Geometry check sheet. Reference: the model listing, model coordinates, mm. Face numbers are marked on the shaded views. A direction names the side the tool comes from. Round coordinates to 2 decimals unless told otherwise and drop trailing zeros. Loops run counter-clockwise (first coordinate to the right, second up) from the corner with the lowest first, then second, coordinate; pieces in that order, holes last. Notation, with made-up numbers: M -27,-34.75 L -12,-34.75 A28 cw -12,-7.75 Z; hole C 45,72.5 d3. An arc over 180 degrees is marked long. Write item = value, one per line.
from build123d import *

# Parameters (mm, degrees)
BOSS_EXTRUDE1_DEPTH                                  = 7.5
SKETCH2_W                                            = 168
SKETCH2_H                                            = 12
CUT_EXTRUDE1_DEPTH                                   = 12
CUT_EXTRUDE2_DEPTH                                   = 489.185415595
SKETCH4_W                                            = 22
SKETCH4_H                                            = 220
CUT_EXTRUDE3_DEPTH                                   = 1.5
F_11_0_11_DIAMETER_HOLE1_D                           = 11
F_11_0_11_DIAMETER_HOLE1_DEPTH                       = 30
SKETCH17_W                                           = 13.5
SKETCH17_H                                           = 16
CUT_EXTRUDE4_DEPTH                                   = 5
M6_TAPPED_HOLE2_D                                    = 5
M6_TAPPED_HOLE2_DEPTH                                = 15
M6_TAPPED_HOLE2_TIP                                  = 1.502151548
M4_TAPPED_HOLE1_D                                    = 3.3
M4_TAPPED_HOLE1_DEPTH                                = 10.1
M4_TAPPED_HOLE1_TIP                                  = 0.991420021
HOLE_SIZE_PER_SOCKET_HEAD_CAP_SCREW_TYPE_D           = 11
HOLE_SIZE_PER_SOCKET_HEAD_CAP_SCREW_TYPE_CBORE_D     = 18
HOLE_SIZE_PER_SOCKET_HEAD_CAP_SCREW_TYPE_CBORE_DEPTH = 11
F_10_0_10_DIAMETER_HOLE1_D                           = 10
F_10_0_10_DIAMETER_HOLE1_DEPTH                       = 30
F_10_0_10_DIAMETER_HOLE1_TIP                         = 3.004303095
M8_TAPPED_HOLE3_D                                    = 6.8
M8_TAPPED_HOLE3_DEPTH                                = 19.75
M8_TAPPED_HOLE3_TIP                                  = 2.042926105
M6_TAPPED_HOLE3_D                                    = 5
M6_TAPPED_HOLE3_DEPTH                                = 15
M6_TAPPED_HOLE3_TIP                                  = 1.502151548
FILLET1_R                                            = 5
M5_TAPPED_HOLE1_D                                    = 4.2
M5_TAPPED_HOLE1_DEPTH                                = 12.4
M5_TAPPED_HOLE1_TIP                                  = 1.2618073
CHAMFER1_SIZE                                        = 1
SKETCH36_OUTSIDE_W                                   = 449.638
SKETCH36_OUTSIDE_H                                   = 439.638
SKETCH36_OUTSIDE_W_2                                 = 200
SKETCH36_OUTSIDE_H_2                                 = 72
CUT_EXTRUDE6_DEPTH                                   = 489.185415598
M4_TAPPED_HOLE2_D                                    = 3.3
M4_TAPPED_HOLE2_DEPTH                                = 10.1
M4_TAPPED_HOLE2_TIP                                  = 0.991420021
HOLE_SIZE_PER_SOCKET_HEAD_CAP_SCREW_2_D              = 5.5
HOLE_SIZE_PER_SOCKET_HEAD_CAP_SCREW_2_CBORE_D        = 9.5
HOLE_SIZE_PER_SOCKET_HEAD_CAP_SCREW_2_CBORE_DEPTH    = 5.7
CHAMFER2_SIZE                                        = 2


with BuildPart() as part:
    # Sketch1 → Boss-Extrude1 (new, symmetric)
    with BuildSketch(Plane.XY):
        Polygon((0, 0), (0, 340), (168, 340), (168, 220), (350, 220), (350, 0), align=None)
    extrude(amount=BOSS_EXTRUDE1_DEPTH, both=True)

    # Sketch2 → Cut-Extrude1 (cut)
    with BuildSketch(Plane(origin=(0, 340, 0), x_dir=(1, 0, 0), z_dir=(0, 1, 0))):
        with Locations((84, 1.5)):
            Rectangle(SKETCH2_W, SKETCH2_H)
    extrude(amount=-CUT_EXTRUDE1_DEPTH, mode=Mode.SUBTRACT)

    # Sketch3 → Cut-Extrude2 (cut, through all)
    with BuildSketch(Plane.XY.offset(7.5)):
        with BuildLine():
            Line((45, 110), (135, 110))
            ThreePointArc((135, 110), (138.535533906, 108.535533906), (140, 105))
            Line((140, 105), (140, 35))
            ThreePointArc((140, 35), (138.535533906, 31.464466094), (135, 30))
            Line((135, 30), (45, 30))
            ThreePointArc((45, 30), (41.464466094, 31.464466094), (40, 35))
            Line((40, 35), (40, 105))
            ThreePointArc((40, 105), (41.464466094, 108.535533906), (45, 110))
        make_face()
        with BuildLine():
            Line((215, 30), (305, 30))
            ThreePointArc((305, 30), (308.535533906, 31.464466094), (310, 35))
            Line((310, 35), (310, 105))
            ThreePointArc((310, 105), (308.535533906, 108.535533906), (305, 110))
            Line((305, 110), (215, 110))
            ThreePointArc((215, 110), (211.464466094, 108.535533906), (210, 105))
            Line((210, 105), (210, 35))
            ThreePointArc((210, 35), (211.464466094, 31.464466094), (215, 30))
        make_face()
    extrude(amount=-CUT_EXTRUDE2_DEPTH, mode=Mode.SUBTRACT)

    # Sketch4 → Cut-Extrude3 (cut)
    with BuildSketch(Plane(origin=(0, 0, -7.5), x_dir=(-1, 0, 0), z_dir=(0, 0, -1))):
        with Locations((-339, 110)):
            Rectangle(SKETCH4_W, SKETCH4_H)
    extrude(amount=-CUT_EXTRUDE3_DEPTH, mode=Mode.SUBTRACT)

    # Ø11.0 (11) Diameter Hole1
    with Locations(Plane(origin=(0, 30, 0), x_dir=(-1, 0, 0), z_dir=(0, 1, 0))):
        with Locations((-285, 0), (-65, 0), (-235, 0), (-115, 0)):
            Hole(F_11_0_11_DIAMETER_HOLE1_D / 2, depth=F_11_0_11_DIAMETER_HOLE1_DEPTH)

    # Sketch17 → Cut-Extrude4 (cut)
    with BuildSketch(Plane(origin=(350, 0, 0), x_dir=(0, 0, -1), z_dir=(1, 0, 0))):
        with Locations((-0.75, 160)):
            Rectangle(SKETCH17_W, SKETCH17_H)
    extrude(amount=-CUT_EXTRUDE4_DEPTH, mode=Mode.SUBTRACT)

    # M6 Tapped Hole2
    with Locations(Plane(origin=(0, 0, -7.5), x_dir=(-1, 0, 0), z_dir=(0, 0, -1))):
        with Locations((-290.5, 15), (-256.5, 15)):
            Hole(M6_TAPPED_HOLE2_D / 2, depth=M6_TAPPED_HOLE2_DEPTH)
            with Locations((0, 0, -(M6_TAPPED_HOLE2_DEPTH + M6_TAPPED_HOLE2_TIP / 2))):  # 118° drill point
                Cone(0, M6_TAPPED_HOLE2_D / 2, M6_TAPPED_HOLE2_TIP, mode=Mode.SUBTRACT)

    # M4 Tapped Hole1
    with Locations(Plane(origin=(0, 0, -6), x_dir=(-1, 0, 0), z_dir=(0, 0, -1))):
        with Locations((-335.5, 200), (-335.5, 140), (-335.5, 80), (-335.5, 20)):
            Hole(M4_TAPPED_HOLE1_D / 2, depth=M4_TAPPED_HOLE1_DEPTH)
            with Locations((0, 0, -(M4_TAPPED_HOLE1_DEPTH + M4_TAPPED_HOLE1_TIP / 2))):  # 118° drill point
                Cone(0, M4_TAPPED_HOLE1_D / 2, M4_TAPPED_HOLE1_TIP, mode=Mode.SUBTRACT)

    # Hole size per socket head cap screw type (through all)
    with Locations(Plane.XY.offset(7.5)):
        with Locations((70, 202), (100, 202), (130, 202), (130, 162), (100, 162), (70, 162)):
            CounterBoreHole(HOLE_SIZE_PER_SOCKET_HEAD_CAP_SCREW_TYPE_D / 2, HOLE_SIZE_PER_SOCKET_HEAD_CAP_SCREW_TYPE_CBORE_D / 2, HOLE_SIZE_PER_SOCKET_HEAD_CAP_SCREW_TYPE_CBORE_DEPTH)

    # Ø10.0 (10) Diameter Hole1
    with Locations(Plane.XY.offset(7.5)):
        with Locations((135, 135), (65, 135)):
            Hole(F_10_0_10_DIAMETER_HOLE1_D / 2, depth=F_10_0_10_DIAMETER_HOLE1_DEPTH)
            with Locations((0, 0, -(F_10_0_10_DIAMETER_HOLE1_DEPTH + F_10_0_10_DIAMETER_HOLE1_TIP / 2))):  # 118° drill point
                Cone(0, F_10_0_10_DIAMETER_HOLE1_D / 2, F_10_0_10_DIAMETER_HOLE1_TIP, mode=Mode.SUBTRACT)

    # M8 Tapped Hole3
    with Locations(Plane(origin=(350, 0, 0), x_dir=(0, 0, -1), z_dir=(1, 0, 0))):
        with Locations((0, 187.5), (0, 132.5)):
            Hole(M8_TAPPED_HOLE3_D / 2, depth=M8_TAPPED_HOLE3_DEPTH)
            with Locations((0, 0, -(M8_TAPPED_HOLE3_DEPTH + M8_TAPPED_HOLE3_TIP / 2))):  # 118° drill point
                Cone(0, M8_TAPPED_HOLE3_D / 2, M8_TAPPED_HOLE3_TIP, mode=Mode.SUBTRACT)

    # M6 Tapped Hole3
    with Locations(Plane(origin=(0, 328, 0), x_dir=(-1, 0, 0), z_dir=(0, 1, 0))):
        with Locations((-151.5, -1.5), (-106.5, -1.5), (-61.5, -1.5), (-16.5, -1.5)):
            Hole(M6_TAPPED_HOLE3_D / 2, depth=M6_TAPPED_HOLE3_DEPTH)
            with Locations((0, 0, -(M6_TAPPED_HOLE3_DEPTH + M6_TAPPED_HOLE3_TIP / 2))):  # 118° drill point
                Cone(0, M6_TAPPED_HOLE3_D / 2, M6_TAPPED_HOLE3_TIP, mode=Mode.SUBTRACT)

    # Fillet1
    fillet1_edges = [part.edges().sort_by_distance(p)[0] for p in [
        (168, 220, 0),
    ]]
    fillet(fillet1_edges, radius=FILLET1_R)

    # M5 Tapped Hole1
    with Locations(Plane(origin=(345, 0, 0), x_dir=(0, 0, -1), z_dir=(1, 0, 0))):
        with Locations((4, 160)):
            Hole(M5_TAPPED_HOLE1_D / 2, depth=M5_TAPPED_HOLE1_DEPTH)
            with Locations((0, 0, -(M5_TAPPED_HOLE1_DEPTH + M5_TAPPED_HOLE1_TIP / 2))):  # 118° drill point
                Cone(0, M5_TAPPED_HOLE1_D / 2, M5_TAPPED_HOLE1_TIP, mode=Mode.SUBTRACT)

    # Chamfer1
    chamfer1_edges = [part.edges().sort_by_distance(p)[0] for p in [
        (0, 0, 0),
        (0, 340, 6),
        (168, 340, 6),
        (350, 220, 0.75),
        (350, 0, 0.75),
    ]]
    chamfer(chamfer1_edges, length=CHAMFER1_SIZE)

    # Sketch36 outside → Cut-Extrude6 (cut, through all)
    with BuildSketch(Plane.XY.offset(7.5)):
        with Locations((175, 170)):
            Rectangle(SKETCH36_OUTSIDE_W, SKETCH36_OUTSIDE_H)
        with Locations((100, 303)):
            Rectangle(SKETCH36_OUTSIDE_W_2, SKETCH36_OUTSIDE_H_2, mode=Mode.SUBTRACT)
    extrude(amount=-CUT_EXTRUDE6_DEPTH, mode=Mode.SUBTRACT)

    # M4 Tapped Hole2
    with Locations(Plane.XY.offset(7.5)):
        with Locations((44, 309.5), (44, 274.5), (124, 274.5), (124, 309.5)):
            Hole(M4_TAPPED_HOLE2_D / 2, depth=M4_TAPPED_HOLE2_DEPTH)
            with Locations((0, 0, -(M4_TAPPED_HOLE2_DEPTH + M4_TAPPED_HOLE2_TIP / 2))):  # 118° drill point
                Cone(0, M4_TAPPED_HOLE2_D / 2, M4_TAPPED_HOLE2_TIP, mode=Mode.SUBTRACT)

    # Hole size per socket head cap screw  2 (through all)
    with Locations(Plane.XY.offset(7.5)):
        with Locations((66.5, 272), (101.5, 272)):
            CounterBoreHole(HOLE_SIZE_PER_SOCKET_HEAD_CAP_SCREW_2_D / 2, HOLE_SIZE_PER_SOCKET_HEAD_CAP_SCREW_2_CBORE_D / 2, HOLE_SIZE_PER_SOCKET_HEAD_CAP_SCREW_2_CBORE_DEPTH)

    # Chamfer2
    chamfer2_edges = [part.edges().sort_by_distance(p)[0] for p in [
        (168, 339, 6),
        (0, 339, 6),
    ]]
    chamfer(chamfer2_edges, length=CHAMFER2_SIZE)


solid = part.part
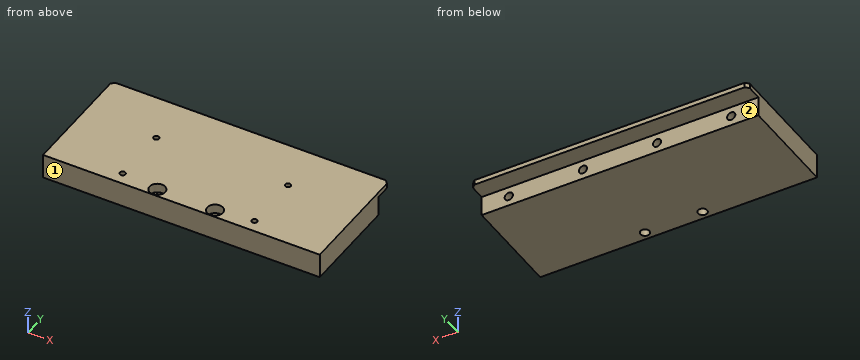
(1) Material ranges on line 1 along Y through (x, z) = (44, 4); line 2 along X through (y, z) = (272, -1.25); line 3 along X through (y, z) = (323, -1.5), recorded low to high. Write a range as from..to.
Result set:
line_1 = 267..272.85, 276.15..307.85, 311.15..328
line_2 = 0..63.75, 69.25..98.75, 104.25..168
line_3 = 0..14, 19..59, 64..104, 109..149, 154..168
(2) Sectioned sample at A-A on x = 66.5. Record the cut outline in (y, z).
Result set:
outline = M 267,-7.5 L 269.25,-7.5 L 269.25,1.8 L 267.25,1.8 L 267.25,7.5 L 267,7.5 Z; M 274.75,-7.5 L 328,-7.5 L 328,4.5 L 339,4.5 L 339,7.5 L 276.75,7.5 L 276.75,1.8 L 274.75,1.8 Z
(3) Tool access check on the marked faces 1 and 2. Record the directions out of +Z, -Z, +X, -X, +Y, -Y that give a thin tool (end or side, any length) a straight path to the whole face; none if there is none.
Result set:
face_1 = +Z, -Z, +X, -X, -Y
face_2 = -Z, +X, -X, +Y
(4) Depth check by flat-ended pin: pin 1 Ø4.5 at (x, z) = (61.5, -1.5) entering from +Y; pin 2 Ø3 at (x, y) = (99.5, 274) entering from +Z; pin 3 Ø2 at (x, z) = (35, 2) entering from +Y. Enter the tip coordinate at first touch or a pass-through.
Result set:
pin_1 = 312.85
pin_2 = 1.8
pin_3 = 328
(5) Sectioned sample at B-B on x = 146. Record the cut outline in (y, z).
Result set:
outline = M 267,-7.5 L 328,-7.5 L 328,4.5 L 339,4.5 L 339,7.5 L 267,7.5 Z
